The listing builds one solid part. Answer for the finished solid, in the listing's coordinates (mm). Coordinates: 2 decimals unless noted, no trailing zeros. Write each loop counter-clockwise with the first axis right and the second up, starting at its lowest first coordinate (ties: lowest second). Pieces come first, ordered by that corner, then holes.
from build123d import *

# Parameters (mm, degrees)
SKETCH1_W           = 8
SKETCH1_H           = 5
BOSS_EXTRUDE1_DEPTH = 0.5
SKETCH2_R           = 1.25
SKETCH2_R_2         = 0.6
CUT_EXTRUDE1_DEPTH  = 5.82182538
CHAMFER1_SIZE       = 0.5


with BuildPart() as part:
    # Sketch1 → Boss-Extrude1 (new, symmetric)
    with BuildSketch(Plane.XY):
        Rectangle(SKETCH1_W, SKETCH1_H)
    extrude(amount=BOSS_EXTRUDE1_DEPTH, both=True)

    # Sketch2 → Cut-Extrude1 (cut, through all)
    with BuildSketch(Plane.XY.offset(0.5)):
        Circle(SKETCH2_R)
        with Locations((-3, 0)):
            Circle(SKETCH2_R_2)
        with Locations((3, 0)):
            Circle(SKETCH2_R_2)
    extrude(amount=-CUT_EXTRUDE1_DEPTH, mode=Mode.SUBTRACT)

    # Chamfer1
    chamfer1_edges = [part.edges().sort_by_distance(p)[0] for p in [
        (4, -2.5, 0),
        (-4, -2.5, 0),
        (-4, 2.5, 0),
        (4, 2.5, 0),
    ]]
    chamfer(chamfer1_edges, length=CHAMFER1_SIZE)


solid = part.part
Q1. The part is cut by section B-B, the plane y = 0. Write down the section's boundary in (x, z).
Answers below:
outline: (-4, -0.5) - (-3.6, -0.5) - (-3.6, 0.5) - (-4, 0.5) - close; (-2.4, -0.5) - (-1.25, -0.5) - (-1.25, 0.5) - (-2.4, 0.5) - close; (1.25, -0.5) - (2.4, -0.5) - (2.4, 0.5) - (1.25, 0.5) - close; (3.6, -0.5) - (4, -0.5) - (4, 0.5) - (3.6, 0.5) - close
Q2. The part is cut by section C-C, the plane z = -0.1. Write down the section's boundary in (x, y).
Answers below:
outline: (-4, -2) - (-3.5, -2.5) - (3.5, -2.5) - (4, -2) - (4, 2) - (3.5, 2.5) - (-3.5, 2.5) - (-4, 2) - close; hole circle Ø1.2 at (-3, 0); hole circle Ø2.5 at (0, 0); hole circle Ø1.2 at (3, 0)
Q3. Determine the mould class of faces 1 (the face through (0, 2.5, 0)), 2 (the face through (4, 0, 0)), 3 (the face through (-3.6, 0, 0)), 4 (the face through (-0.27, -1.22, 0.01)) for opening direction X: released by +X, released by -X, zero draft, split by the parting line, or undercut.
Answers below:
face 1: zero draft
face 2: released by +X
face 3: undercut
face 4: undercut
Q4. The part is cut by section D-D, the plane x = 3. Write down the section's boundary in (y, z), then the cut area to 3 significant figures.
Answers below:
outline: (-2.5, -0.5) - (-0.6, -0.5) - (-0.6, 0.5) - (-2.5, 0.5) - close; (0.6, -0.5) - (2.5, -0.5) - (2.5, 0.5) - (0.6, 0.5) - close
area: 3.80 mm2
Q5. Find the intervals of material crossed by probe 1 along Y at (x, z) = (-3, -0.3); probe 2 along X at (y, z) = (-0.25, 0.45); probe 3 along X at (y, z) = (-0.15, 0), in increasing order.
Answers below:
probe 1: y = -2.5 to -0.6, 0.6 to 2.5
probe 2: x = -4 to -3.55, -2.45 to -1.22, 1.22 to 2.45, 3.55 to 4
probe 3: x = -4 to -3.58, -2.42 to -1.24, 1.24 to 2.42, 3.58 to 4
Q6. The part is cut by section A-A, the plane x = 0. Write down the section's boundary in (y, z), then the cut area to 3 significant figures.
Answers below:
outline: (-2.5, -0.5) - (-1.25, -0.5) - (-1.25, 0.5) - (-2.5, 0.5) - close; (1.25, -0.5) - (2.5, -0.5) - (2.5, 0.5) - (1.25, 0.5) - close
area: 2.50 mm2
